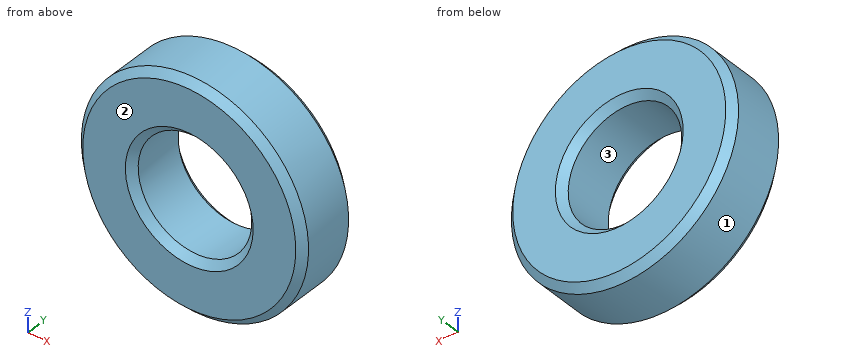
from build123d import *

# Parameters (mm, degrees)
SKETCH1_R           = 8
SKETCH1_R_2         = 4
BOSS_EXTRUDE1_DEPTH = 4.5
CHAMFER1_SIZE       = 0.5


with BuildPart() as part:
    # Sketch1 → Boss-Extrude1 (new body)
    with BuildSketch(Plane(origin=(0, 0, 0), x_dir=(1, 0, 0), z_dir=(0, 1, 0))):
        with Locations(Location((0, 0, 0), (0, 0, 270))):
            Circle(SKETCH1_R)
        with Locations(Location((0, 0, 0), (0, 0, 270))):
            Circle(SKETCH1_R_2, mode=Mode.SUBTRACT)
    extrude(amount=BOSS_EXTRUDE1_DEPTH)

    # Chamfer1
    chamfer1_edges = [part.edges().sort_by_distance(p)[0] for p in [
        (0, 0, -8),
        (0, 4.5, -8),
        (0, 0, -4),
        (0, 4.5, -4),
    ]]
    chamfer(chamfer1_edges, length=CHAMFER1_SIZE)


solid = part.part
Verification items for the finished model (mm, model axes). Face numbers are marked on the shaded views. Coordinates: 2 decimals unless noted, no trailing zeros. Order: outer loops, then holes, each group sorted by start corner. A loop starts at its lowest first (then second) coordinate and runs counter-clockwise, first axis right, second up. Notation, with made-up numbers: (70.25, 8) -> (84.25, 8) arc R15 ccw to (84.25, 22) -> close; hole circle Ø6 at (-35, 70.5). An arc over 180 degrees is marked (long way). Put each result on its own line as item: value. Start each with the question number.
1. Cross-section at C-C, the plane y = 0.95. Record the boundary of the cut face in (x, z).
2. Mould release check, pull along Z, two halves, no side actions. Record for the marked faces 1, 2 and 3: released by +Z, released by -Z, zero draft, split by the parting line, or undercut.
3. Cross-section at B-B, the plane x = 0. Record the boundary of the cut face in (y, z), then the cut area to 3 significant figures.
4. Material ranges on L1, parallel to X at y = 1.85, z = 0; L2, parallel to Z at x = -2.5, y = 3.5; L3, parallel to Z at x = 7, y = 2.1, recorded low to high. Write a range as [from, to].
5. Cross-section at A-A, the plane z = 0. Record the boundary of the cut face in (x, y).
6. Go/stop test with flat-tipped pins: pin 1 Ø1.5 at (y, z) = (3.5, 1.5) entering from -X; pin 2 Ø1 at (x, y) = (3, 2) entering from +Z. Record where each tip stops, or that it passes through.
Computed:
1. outline: circle Ø16 at (0, 0); hole circle Ø8 at (0, 0)
2. face 1: split by the parting line
2. face 2: zero draft
2. face 3: undercut
3. outline: (0, -7.5) -> (0.5, -8) -> (4, -8) -> (4.5, -7.5) -> (4.5, -4.5) -> (4, -4) -> (0.5, -4) -> (0, -4.5) -> close; (0, 4.5) -> (0.5, 4) -> (4, 4) -> (4.5, 4.5) -> (4.5, 7.5) -> (4, 8) -> (0.5, 8) -> (0, 7.5) -> close
3. area: 35.0 mm2
4. L1: [-8, -4], [4, 8]
4. L2: [-7.6, -3.12], [3.12, 7.6]
4. L3: [-3.87, 3.87]
5. outline: (-8, 0.5) -> (-7.5, 0) -> (-4.5, 0) -> (-4, 0.5) -> (-4, 4) -> (-4.5, 4.5) -> (-7.5, 4.5) -> (-8, 4) -> close; (4, 0.5) -> (4.5, 0) -> (7.5, 0) -> (8, 0.5) -> (8, 4) -> (7.5, 4.5) -> (4.5, 4.5) -> (4, 4) -> close
6. pin 1: x = -7.96
6. pin 2: z = 7.6
